from build123d import *

# Parameters (mm, degrees)
SKETCH1_W           = 50
SKETCH1_H           = 30
BOSS_EXTRUDE1_DEPTH = 3
SKETCH2_R           = 2.5
BOSS_EXTRUDE2_DEPTH = 85
SKETCH3_W           = 10
SKETCH3_H           = 12
BOSS_EXTRUDE3_DEPTH = 22
SKETCH4_W           = 17.596186584
SKETCH4_H           = 6
CUT_EXTRUDE1_DEPTH  = 20
SKETCH5_R           = 2.5
CUT_EXTRUDE2_DEPTH  = 115.743191519


with BuildPart() as part:
    # Sketch1 → Boss-Extrude1 (new body)
    with BuildSketch(Plane.XY):
        Rectangle(SKETCH1_W, SKETCH1_H)
    extrude(amount=BOSS_EXTRUDE1_DEPTH)

    # Sketch2 → Boss-Extrude2 (add)
    with BuildSketch(Plane.XY.offset(3)):
        Circle(SKETCH2_R)
    extrude(amount=BOSS_EXTRUDE2_DEPTH)

    # Sketch3 → Boss-Extrude3 (add)
    with BuildSketch(Plane.XY.offset(88)):
        Rectangle(SKETCH3_W, SKETCH3_H)
    extrude(amount=BOSS_EXTRUDE3_DEPTH)

    # Sketch4 → Cut-Extrude1 (cut)
    with BuildSketch(Plane.XY.offset(110)):
        Rectangle(SKETCH4_W, SKETCH4_H)
    extrude(amount=-CUT_EXTRUDE1_DEPTH, mode=Mode.SUBTRACT)

    # Sketch5 → Cut-Extrude2 (cut, through all)
    with BuildSketch(Plane(origin=(0, -6, 0), x_dir=(-1, 0, 0), z_dir=(0, -1, 0))):
        with Locations(Location((0, -105, 0), (0, 0, 90))):
            Circle(SKETCH5_R)
        with BuildLine():
            Line((5, -105), (16.865416132, -140.325641039))
            Line((16.865416132, -140.325641039), (-16.120021854, -140.325641039))
            Line((-16.120021854, -140.325641039), (-5, -105))
            ThreePointArc((-5, -105), (0, -110), (5, -105))
        make_face()
    extrude(amount=-CUT_EXTRUDE2_DEPTH, mode=Mode.SUBTRACT)


solid = part.part
The model under review builds one solid part; all positions refer to its coordinate system, in mm. A direction names the side the tool comes from. Round coordinates to 2 decimals unless told otherwise and drop trailing zeros. Loops run counter-clockwise (first coordinate to the right, second up) from the corner with the lowest first, then second, coordinate; pieces in that order, holes last. Notation, with made-up numbers: M 75.25,62 L 96.25,62 A27 cw 96.25,92 Z; hole C 63.25,6 d4. An arc over 180 degrees is marked long. Answer as a JSON object with one key per item and string values.
Item 1: We need section A-A, the plane z = 93. State the section outline as (x, y) points.
Check sheet entries:
{"outline": "M -5,-6 L 5,-6 L 5,-3 L -5,-3 Z; M -5,3 L 5,3 L 5,6 L -5,6 Z"}
Item 2: The part is to be moulded in two halves that separate along Z. For faces 5 (the face through (0, -6, 99)), 6 (the face through (0.751, -4.521, 102.615)), 7 (the face through (-0.54, -2.44, 44.9)), 8 (the face through (0, 4, 110)), say which applies: +Z half, -Z half, draft (parallel to the pull), parting line (faces both ways), or undercut.
Check sheet entries:
{"face 5": "draft", "face 6": "undercut", "face 7": "undercut", "face 8": "+Z half"}
Item 3: We need section C-C, the plane x = 20. State the section outline as (y, z) points, and give its area (3 significant figures).
Check sheet entries:
{"outline": "M -15,0 L 15,0 L 15,3 L -15,3 Z", "area": "90.0 mm2"}
Item 4: Clearance check with flat-ended pins moving along their axes: P1, Ø1.5, axis at x = 18, y = 3.5, coming from the +Z side; P2, Ø5, axis at x = -9, y = -1.5, coming from the -Z side; P3, Ø6, axis at y = 0.5, z = 94, coming from the -X side; P4, Ø9, axis at x = 4.5, y = -1.5, coming from the +Z side. State where each tip first meets the part, or that it passes through.
Check sheet entries:
{"P1": "z = 3", "P2": "z = 0", "P3": "x = -5", "P4": "z = 109.99"}
Item 5: For line 1 along X through (y, z) = (-4.6, 105); line 2 along Z through (x, y) = (-19, -3.75); line 3 along Y through (x, z) = (0, 56), list the stretches that pass through material, from the lowest coordinate up.
Check sheet entries:
{"line 1": "-5 to -2.5, 2.5 to 5", "line 2": "0 to 3", "line 3": "-2.5 to 2.5"}
Item 6: Tool access review of faces 1 (the face through (-5, -4, 96)), 2 (the face through (5, -4, 96)), 3 (the face through (0, 0, 90)), 4 (the face through (0, 6, 99)): name each direction out of +Z, -Z, +X, -X, +Y, -Y from which nothing blocks a thin tool from reaching the whole face with its end or side.
Check sheet entries:
{"face 1": "+Z, -X, +Y, -Y", "face 2": "+Z, +X, +Y, -Y", "face 3": "+Z, +X, -X", "face 4": "+Z, +X, -X, +Y"}
Item 7: We need section D-D, the plane z = 70. State the section outline as (x, y) points, and give its area (3 significant figures).
Check sheet entries:
{"outline": "C 0,0 d5", "area": "19.6 mm2"}
Item 8: We need section B-B, the plane y = 0. State the section outline as (x, z) points.
Check sheet entries:
{"outline": "M -25,0 L 25,0 L 25,3 L 2.5,3 L 2.5,88 L 5,88 L 5,90 L -5,90 L -5,88 L -2.5,88 L -2.5,3 L -25,3 Z"}
